```python
from build123d import *

# Parameters (mm, degrees)
SKETCH1_R           = 250
BOSS_EXTRUDE1_DEPTH = 3
SKETCH2_R           = 77
CUT_EXTRUDE1_DEPTH  = 10
CIRPATTERN1_COUNT   = 4


with BuildPart() as part:
    # Sketch1 → Boss-Extrude1 (new body)
    with BuildSketch(Plane(origin=(0, 0, 0), x_dir=(0, 0, -1), z_dir=(1, 0, 0))):
        Circle(SKETCH1_R)
    extrude(amount=BOSS_EXTRUDE1_DEPTH)

    # Sketch2 → Cut-Extrude1 (cut)
    with BuildSketch(Plane(origin=(3, 0, 0), x_dir=(0, 0, -1), z_dir=(1, 0, 0))):
        with Locations((0, 125)):
            Circle(SKETCH2_R)
    cut_extrude1 = extrude(amount=-CUT_EXTRUDE1_DEPTH, mode=Mode.SUBTRACT)

    # CirPattern1: Cut-Extrude1 ×4 about axis
    cirpattern1_axis = Axis((0, 0, 0), (1, 0, 0))
    for i in range(1, CIRPATTERN1_COUNT):
        add(cut_extrude1.rotate(cirpattern1_axis, i * 360 / CIRPATTERN1_COUNT), mode=Mode.SUBTRACT)


solid = part.part
```
CAD build for the part. Positions are in the model's coordinates, mm. Coordinates: 2 decimals unless noted, no trailing zeros. Loops run counter-clockwise (first coordinate to the right, second up) from the corner with the lowest first, then second, coordinate; pieces in that order, holes last. Notation, with made-up numbers: (-9.5, 79.25) - (46.5, 79.25) arc R21 cw to (46.5, 98.25) - close; hole circle Ø9 at (-16, 52.5). An arc over 180 degrees is marked (long way). Use CSV: the item, a comma, the result in double quotes. Start each with the question number.
Q1. Cut at B-B, the plane y = 16. List the corners of the cut face in (x, z), then the cut area to 3 significant figures.
Q2. Drop flat-ended pins along their axis: P1, Ø1.5, axis at x = 0.5, z = 175.5, coming from the -Y side; P2, Ø1.5, axis at y = -106.5, z = 186, coming from the -X side. Give the stop position or say it passes through.
Q3. Cut at C-C, the plane x = 2.45. List the corners of the cut face in (y, z), then the cut area to 3 significant figures.
Q4. Cut at D-D, the plane z = 194.5. List the corners of the cut face in (x, y).
Q5. Two-plate mould, pull along Y, no slides. Class faces 1 (the flat face through (0, 4, 3)), 2 (the cylindrical face through (1.48, 10.99, 249.76)), 3 (the cylindrical face through (1.52, 49.83, 16.69)): +Y half, -Y half, draft (parallel to the pull), parting line (faces both ways), or undercut.
Q6. Cut at A-A, the plane z = 0. List the corners of the cut face in (x, y), then the cut area to 3 significant figures.
Q7. Probe probe 1 along Y at (x, z) = (1.35, 0); probe 2 along Z at (x, y) = (2, -58); probe 3 along Y at (x, z) = (2.8, -31). List the from-to ranges inside material, lowest first. Write a range as from..to.
Here are the results:
1,outline,"(0, -249.49) - (3, -249.49) - (3, -200.32) - (0, -200.32) - close; (0, -49.68) - (3, -49.68) - (3, 49.68) - (0, 49.68) - close; (0, 200.32) - (3, 200.32) - (3, 249.49) - (0, 249.49) - close"
1,area,"593 mm2"
2,P1,"y = -178.78"
2,P2,"x = 0"
3,outline,"circle Ø500 at (0, 0); hole circle Ø154 at (-125, 0); hole circle Ø154 at (0, -125); hole circle Ø154 at (0, 125); hole circle Ø154 at (125, 0)"
3,area,"122,000 mm2"
4,outline,"(0, -157.07) - (3, -157.07) - (3, -33.15) - (0, -33.15) - close; (0, 33.15) - (3, 33.15) - (3, 157.07) - (0, 157.07) - close"
5,face 1,"draft"
5,face 2,"parting line"
5,face 3,"undercut"
6,outline,"(0, -250) - (3, -250) - (3, -202) - (0, -202) - close; (0, -48) - (3, -48) - (3, 48) - (0, 48) - close; (0, 202) - (3, 202) - (3, 250) - (0, 250) - close"
6,area,"576 mm2"
7,probe 1,"-250..-202, -48..48, 202..250"
7,probe 2,"-243.18..-175.65, -74.35..-37.95, 37.95..74.35, 175.65..243.18"
7,probe 3,"-248.07..-195.48, -54.52..54.52, 195.48..248.07"
